Model file for the job. Use its own axes, mm. A direction names the side the tool comes from. Round coordinates to 2 decimals unless told otherwise and drop trailing zeros. Order: outer loops, then holes, each group sorted by start corner. A loop starts at its lowest first (then second) coordinate and runs counter-clockwise, first axis right, second up. Notation, with made-up numbers: (49, -37.5) -> (96, -37.5) arc R27 cw to (96, -18.5) -> close; hole circle Ø4 at (-13.75, 82.25). An arc over 180 degrees is marked (long way). Put each result on its own line as item: value. Start each with the question number.
Q1. Probe L1, parallel to X at y = 10, z = 6; L2, parallel to Y at x = 6.75, z = 180.5; L3, parallel to Y at x = 3.7, z = 50.5. List the from-to ranges inside material, lowest first.
Q2. Flat gauge pins, fed straight in: P1, Ø2, axis at x = 5, y = 2.5, coming from the -Z side; P2, Ø4, axis at x = 4, z = 14, coming from the -Y side; P3, Ø4.5, axis at x = 6, y = 2, coming from the -Z side. Where does each tip first touch, or does it go through?
Q3. Pull direction Y, two halves, no side cores. Call faces 1 (the face through (4.6, 4, 49)), 2 (the face through (4.6, 4, 59)), 3 (the face through (2.9, 9, 120)), 4 (the face through (1.5, 8.1, 120.6)): released by +Y, released by -Y, zero draft, split by the parting line, or undercut.
Q4. Cut at A-A, the plane y = 14. List the corners of the cut face in (x, z), and give its area (3 significant figures).
Q5. Cut at B-B, the plane z = 221.5. List the corners of the cut face in (x, y), and give its area (3 significant figures).
Q6. 3-axis set-ups, long thin cutter, end or side, ignore diameter. For faces 5 (the face through (4, 5, 229)), 6 (the face through (5, 2, 112.5)), 7 (the face through (6.324, 2.838, 189.116)): which of +Z, -Z, +X, -X, +Y, -Y reach the whole face in a straight line?
from build123d import *

# Parameters (mm, degrees)
SKETCH3_W                                            = 8
SKETCH3_H                                            = 16
BOSS_EXTRUDE2_DEPTH                                  = 241
CUT_EXTRUDE1_DEPTH                                   = 5.1
CUT_EXTRUDE2_DEPTH                                   = 242.584374495
CBORE_FOR_M3_HEXAGON_SOCKET_HEAD_CAP_SCR_D           = 3.4
CBORE_FOR_M3_HEXAGON_SOCKET_HEAD_CAP_SCR_DEPTH       = 10.1
CBORE_FOR_M3_HEXAGON_SOCKET_HEAD_CAP_SCR_CBORE_D     = 6
CBORE_FOR_M3_HEXAGON_SOCKET_HEAD_CAP_SCR_CBORE_DEPTH = 3.4
CBORE_FOR_M3_HEXAGON_SOCKET_HEAD_CAP_SCR_TIP         = 1.021463052
M4_TAPPED_HOLE1_D                                    = 3.3
M4_TAPPED_HOLE1_DEPTH                                = 9.1
M4_TAPPED_HOLE1_TIP                                  = 0.991420021
CUT_EXTRUDE3_DEPTH                                   = 242.662988478


with BuildPart() as part:
    # Sketch3 → Boss-Extrude2 (new body)
    with BuildSketch(Plane.XY):
        with Locations((4, 8)):
            Rectangle(SKETCH3_W, SKETCH3_H)
    extrude(amount=BOSS_EXTRUDE2_DEPTH)

    # Sketch4 → Cut-Extrude1 (cut)
    with BuildSketch(Plane(origin=(8, 0, 0), x_dir=(0, 0, -1), z_dir=(1, 0, 0))):
        with BuildLine():
            Line((-112.5, 4), (-112.5, 0))
            ThreePointArc((-112.5, 0), (-120.5, -8), (-128.5, 0))
            Line((-128.5, 0), (-128.5, 4))
            ThreePointArc((-128.5, 4), (-120.5, 12), (-112.5, 4))
        make_face()
    extrude(amount=-CUT_EXTRUDE1_DEPTH, mode=Mode.SUBTRACT)

    # Sketch5 → Cut-Extrude2 (cut, through all)
    with BuildSketch(Plane(origin=(2.9, 0, 0), x_dir=(0, 0, -1), z_dir=(1, 0, 0))):
        with BuildLine():
            Line((-116.4, 4), (-116.4, 0))
            ThreePointArc((-116.4, 0), (-120.5, -4.1), (-124.6, 0))
            Line((-124.6, 0), (-124.6, 4))
            ThreePointArc((-124.6, 4), (-120.5, 8.1), (-116.4, 4))
        make_face()
    extrude(amount=-CUT_EXTRUDE2_DEPTH, mode=Mode.SUBTRACT)

    # CBORE for M3 Hexagon socket head cap screws1
    with Locations(Plane(origin=(8, 0, 0), x_dir=(0, 0, -1), z_dir=(1, 0, 0))):
        with Locations((-60.5, 5.5), (-50.5, 5.5), (-190.5, 5.5), (-180.5, 5.5)):
            CounterBoreHole(CBORE_FOR_M3_HEXAGON_SOCKET_HEAD_CAP_SCR_D / 2, CBORE_FOR_M3_HEXAGON_SOCKET_HEAD_CAP_SCR_CBORE_D / 2, CBORE_FOR_M3_HEXAGON_SOCKET_HEAD_CAP_SCR_CBORE_DEPTH, depth=CBORE_FOR_M3_HEXAGON_SOCKET_HEAD_CAP_SCR_DEPTH)
            with Locations((0, 0, -(CBORE_FOR_M3_HEXAGON_SOCKET_HEAD_CAP_SCR_DEPTH + CBORE_FOR_M3_HEXAGON_SOCKET_HEAD_CAP_SCR_TIP / 2))):  # 118° drill point
                Cone(0, CBORE_FOR_M3_HEXAGON_SOCKET_HEAD_CAP_SCR_D / 2, CBORE_FOR_M3_HEXAGON_SOCKET_HEAD_CAP_SCR_TIP, mode=Mode.SUBTRACT)

    # M4 Tapped Hole1
    with Locations(Plane(origin=(0, 16, 0), x_dir=(1, 0, 0), z_dir=(0, 1, 0))):
        with Locations((4, -235), (4, -227), (4, -14), (4, -6)):
            Hole(M4_TAPPED_HOLE1_D / 2, depth=M4_TAPPED_HOLE1_DEPTH)
            with Locations((0, 0, -(M4_TAPPED_HOLE1_DEPTH + M4_TAPPED_HOLE1_TIP / 2))):  # 118° drill point
                Cone(0, M4_TAPPED_HOLE1_D / 2, M4_TAPPED_HOLE1_TIP, mode=Mode.SUBTRACT)

    # Sketch10 → Cut-Extrude3 (cut, through all)
    with BuildSketch(Plane(origin=(8, 0, 0), x_dir=(0, 0, -1), z_dir=(1, 0, 0))):
        with BuildLine():
            Line((0, 0), (-25, 0))
            Line((-25, 0), (-25, 3))
            ThreePointArc((-25, 3), (-24.414213562, 4.414213562), (-23, 5))
            Line((-23, 5), (0, 5))
            Line((0, 5), (0, 0))
        make_face()
        with BuildLine():
            Line((-216, 0), (-216, 3))
            ThreePointArc((-216, 3), (-216.585786438, 4.414213562), (-218, 5))
            Line((-218, 5), (-241, 5))
            Line((-241, 5), (-241, 0))
            Line((-241, 0), (-216, 0))
        make_face()
    extrude(amount=-CUT_EXTRUDE3_DEPTH, mode=Mode.SUBTRACT)


solid = part.part
Ans:
1. L1: x = 0 to 2.35, 5.65 to 8
1. L2: y = 0 to 2.5, 8.5 to 16
1. L3: y = 0 to 3.8, 7.2 to 16
2. P1: stops at z = 24.94
2. P2: stops at y = 5
2. P3: stops at z = 24.56
3. face 1: undercut
3. face 2: undercut
3. face 3: zero draft
3. face 4: released by -Y
4. outline: (0, 0) -> (8, 0) -> (8, 241) -> (0, 241) -> close; hole circle Ø3.3 at (4, 6); hole circle Ø3.3 at (4, 14); hole circle Ø3.3 at (4, 227); hole circle Ø3.3 at (4, 235)
4. area: 1,890 mm^2
5. outline: (0, 5) -> (8, 5) -> (8, 16) -> (0, 16) -> close
5. area: 88.0 mm^2
6. face 5: +Z, +X, -X, -Y
6. face 6: +X, -Y
6. face 7: +X
